Source: CAD feature listing. Evaluate the final solid. Frame: model axes, mm. Face numbers are marked on the shaded views. A direction names the side the tool comes from. Give positions to 0.01 mm unless a question says otherwise; leave off trailing zeros. Write each loop counter-clockwise with the first axis right and the second up, starting at its lowest first coordinate (ties: lowest second). Pieces come first, ordered by that corner, then holes. Notation, with made-up numbers: (44.25, 37) - (95.25, 37) arc R20 cw to (95.25, 70) - close; hole circle Ø3 at (-26, 72). An arc over 180 degrees is marked (long way). Answer as a JSON object with one key per item and string values. Group by question number.
from build123d import *

# Parameters (mm, degrees)
BOSS_EXTRUDE1_DEPTH      = 4.7625
BOSS_EXTRUDE1_DEPTH_BACK = 4.7625
SKETCH1_R                = 3.9624
BOSS_EXTRUDE2_DEPTH      = 9.525
BOSS_EXTRUDE2_DEPTH_BACK = 9.525
BOSS_EXTRUDE2_START      = -4.7625
SKETCH2_R                = 3.175


with BuildPart() as part:
    # Sketch1 → Boss-Extrude1 (new, two sides: drawn at the far end of the back side and taken through both)
    with BuildSketch(Plane.XY.offset(-BOSS_EXTRUDE1_DEPTH_BACK)):
        Circle(SKETCH1_R)
    extrude(amount=BOSS_EXTRUDE1_DEPTH + BOSS_EXTRUDE1_DEPTH_BACK)

    # Sketch2 → Boss-Extrude2 (add, two sides: drawn at the far end of the back side and taken through both)
    with BuildSketch(Plane.XY.offset(4.7625).offset(BOSS_EXTRUDE2_START - BOSS_EXTRUDE2_DEPTH_BACK)):
        Circle(SKETCH2_R)
    extrude(amount=BOSS_EXTRUDE2_DEPTH + BOSS_EXTRUDE2_DEPTH_BACK)


solid = part.part
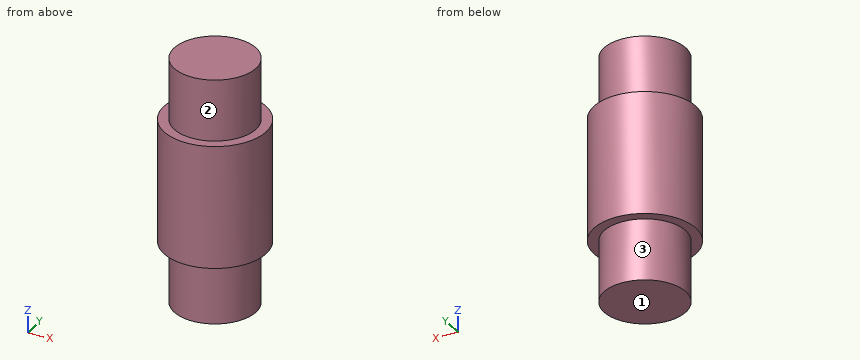
Q1. First-contact query: pin 1 Ø1.5 at (y, z) = (3, -7.5) entering from +X; pin 2 Ø3 at (x, z) = (-2, -1.5) entering from +Y; pin 3 Ø1 at (x, z) = (-0.5, -2.5) entering from +Y. Flat tips, straight axial feed; report the tip coordinate or a pass-through.
Q2. Section A-A on x = 0. Return the cut outline in (y, z) (1 decimal), then the cut area to 3 significant figures.
Q3. Section C-C on z = 1.5. Return the cut outline in (x, y).
Q4. Ray query, probe 1 along Z at (x, y) = (-2.5, 2.25); probe 2 along Y at (x, z) = (0, 5.75) (3 decimals); probe 3 along X at (y, z) = (-2.5, 6.5). Return the intervals inside material, ascending. Write a range as [from, to].
Q5. Section D-D on z = -5.25. Return the cut outline in (x, y) (3 decimals), then the cut area to 3 significant figures.
Q6. Reachability of the marked faces 1, 2 and 3 from +Z, -Z, +X, -X, +Y, -Y: full face, straight path, thin tool, end or side. Return the list, or none.
Taken from the geometry:
{
 "1": {"pin 1": "stops at x = 2.24", "pin 2": "stops at y = 3.93", "pin 3": "stops at y = 3.96"},
 "2": {"outline": "(-4, -4.8) - (-3.2, -4.8) - (-3.2, -9.5) - (3.2, -9.5) - (3.2, -4.8) - (4, -4.8) - (4, 4.8) - (3.2, 4.8) - (3.2, 9.5) - (-3.2, 9.5) - (-3.2, 4.8) - (-4, 4.8) - close", "area": "136 mm²"},
 "3": {"outline": "circle Ø7.92 at (0, 0)"},
 "4": {"probe 1": "z = [-4.76, 4.76]", "probe 2": "y = [-3.175, 3.175]", "probe 3": "x = [-1.96, 1.96]"},
 "5": {"outline": "circle Ø6.35 at (0, 0)", "area": "31.7 mm²"},
 "6": {"face 1": "-Z, +X, -X, +Y, -Y", "face 2": "+Z", "face 3": "-Z"}
}
